```python
from build123d import *

# Parameters (mm, degrees)
HOLE_WIZARD_M5_1_D = 4.2
CHAMFER_1_SIZE     = 0.3


with BuildPart() as part:
    # 草图1 → 旋转1 (revolve)
    with BuildSketch(Plane.XY, mode=Mode.PRIVATE) as revolve_1_sk:
        Polygon((0, 6.5), (-5, 6.5), (-5, 2), (-3.975, 2), (-3.975, 0), (-3.25, 0), (-3.25, 2), (0, 2), align=None)
    revolve(revolve_1_sk.sketch.rotate(Axis((0, 0, 0), (0, 1, 0)), 270), axis=Axis((0, 0, 0), (0, 1, 0)))

    # M5 螺纹孔1 (through all)
    with Locations(Plane(origin=(0, 6.5, 0), x_dir=(1, 0, 0), z_dir=(0, 1, 0))):
        with Locations((0, 0)):
            Hole(HOLE_WIZARD_M5_1_D / 2)

    # 倒角1
    chamfer_1_edges = [part.edges().sort_by_distance(p)[0] for p in [
        (2.1, 2, 0),
        (2.1, 6.5, 0),
        (0, 6.5, 5),
    ]]
    chamfer(chamfer_1_edges, length=CHAMFER_1_SIZE)


solid = part.part
```
Build history of the part. All positions in model axes, mm. Round coordinates to 2 decimals unless told otherwise and drop trailing zeros. Write each loop counter-clockwise with the first axis right and the second up, starting at its lowest first coordinate (ties: lowest second). Pieces come first, ordered by that corner, then holes. Notation, with made-up numbers: (58.5, 83.25) -> (102.5, 83.25) arc R21 ccw to (102.5, 104.25) -> close; hole circle Ø8 at (-19.75, 61.5). An arc over 180 degrees is marked (long way). Put each result on its own line as item: value.
Item 1: Slice it at B-B, the plane x = 0. Give the cut face in (y, z) (3 decimals).
Here are the results:
outline: (0, -3.975) -> (2, -3.975) -> (2, -5) -> (6.2, -5) -> (6.5, -4.7) -> (6.5, -2.4) -> (6.2, -2.1) -> (2.3, -2.1) -> (2, -2.4) -> (2, -3.25) -> (0, -3.25) -> close; (0, 3.25) -> (2, 3.25) -> (2, 2.4) -> (2.3, 2.1) -> (6.2, 2.1) -> (6.5, 2.4) -> (6.5, 4.7) -> (6.2, 5) -> (2, 5) -> (2, 3.975) -> (0, 3.975) -> close
Item 2: Two-plate mould, pull along X, no slides. Class faces 1 (the face through (4, 2, 2)), 2 (the face through (2.419, 0.986, 3.154)), 3 (the face through (1.978, 1.014, 2.579)): pulls with the +X half, pulls with the -X half, needs draft (parallel to the pull), parting line crosses it, or undercut.
Here are the results:
face 1: needs draft
face 2: parting line crosses it
face 3: undercut
Item 3: Slice it at C-C, the plane y = 1.25. Give the cut face in (x, z) (3 decimals), plus the area to 3 significant figures.
Here are the results:
outline: circle Ø7.95 at (0, 0); hole circle Ø6.5 at (0, 0)
area: 16.5 mm^2
Item 4: Slice it at D-D, the plane y = 6. Give the cut face in (x, z), plus the area to 3 significant figures.
Here are the results:
outline: circle Ø10 at (0, 0); hole circle Ø4.2 at (0, 0)
area: 64.7 mm^2
Item 5: Slice it at A-A, the plane z = 0. Give the cut face in (x, y) (3 decimals), plus the area to 3 significant figures.
Here are the results:
outline: (-5, 2) -> (-3.975, 2) -> (-3.975, 0) -> (-3.25, 0) -> (-3.25, 2) -> (-2.4, 2) -> (-2.1, 2.3) -> (-2.1, 6.2) -> (-2.4, 6.5) -> (-4.7, 6.5) -> (-5, 6.2) -> close; (2.1, 2.3) -> (2.4, 2) -> (3.25, 2) -> (3.25, 0) -> (3.975, 0) -> (3.975, 2) -> (5, 2) -> (5, 6.2) -> (4.7, 6.5) -> (2.4, 6.5) -> (2.1, 6.2) -> close
area: 28.7 mm^2
Item 6: Wall check: probe 1 along X at (y, z) = (3.65, 0); probe 2 along Y at (x, z) = (4.25, 0.75); probe 3 along X at (y, z) = (0.4, 0) (3 decimals). Give the ranges that are in metal, low to high. Write a range as from..to.
Here are the results:
probe 1: x = -5..-2.1, 2.1..5
probe 2: y = 2..6.5
probe 3: x = -3.975..-3.25, 3.25..3.975
Item 7: Flat gauge pins, fed straight in: P1, Ø2, axis at x = -2.5, y = 4, coming from the -Z side; P2, Ø1.5, axis at y = 2.5, z = -4, coming from the -X side; P3, Ø1.5, axis at y = 2.5, z = 2.5, coming from the -X side; P4, Ø2, axis at x = -1, z = 0, coming from the -Y side. Where does each tip first touch, or does it go through?
Here are the results:
P1: stops at z = -4.77
P2: stops at x = -3.8
P3: stops at x = -4.68
P4: passes through
